Input: dimensioned drawing with shaded views. Units: mm. Origin: part minimum x, y, z. A direction names the side the tool comes from. Coordinates: 2 decimals unless noted, no trailing zeros. Write each loop counter-clockwise with the first axis right and the second up, starting at its lowest first coordinate (ties: lowest second). Pieces come first, ordered by that corner, then holes. Notation, with made-up numbers: (58.25, 23) -> (68.25, 23) arc R14 ccw to (68.25, 38) -> close; hole circle Ø7 at (19.5, 54). An arc over 180 degrees is marked (long way). One line per item, written item: value. Start each with the question number.
1. Line query: line 1 (X direction, y = 12, z = 9.75); line 2 (X direction, y = 2.25, z = 8.5); line 3 (Z direction, x = 23, y = 12.25). Output: solid intervals per line, ascending.
2. Access query for the marked faces 1 and 2. Directions: +Z, -Z, +X, -X, +Y, -Y. A direction counts if a zero-diameter tool reaches every point of the face in a straight line with its end or side. Return the directions, or none.
3. Section query B-B, the plane z = 12. Output: boundary loops of the cut face in (x, y), and give its area (3 significant figures).
4. Section query D-D, the plane x = 72. Output: boundary loops of the cut face in (y, z), and give its area (3 significant figures).
5. Section query C-C, the plane x = 102. Output: boundary loops of the cut face in (y, z), and give its area (3 significant figures).
6. Section query A-A, the plane y = 12. Output: boundary loops of the cut face in (x, z), and give its area (3 significant figures).
7. First-contact query: P1, Ø10, axis at x = 99, z = 17, coming from the +Y side; P2, Ø5, axis at x = 64.5, y = 11.5, coming from the -Z side; P3, Ø1.5, axis at x = 71.5, y = 6, coming from the +Z side. Flat tips, straight axial feed; report the tip coordinate or a pass-through.
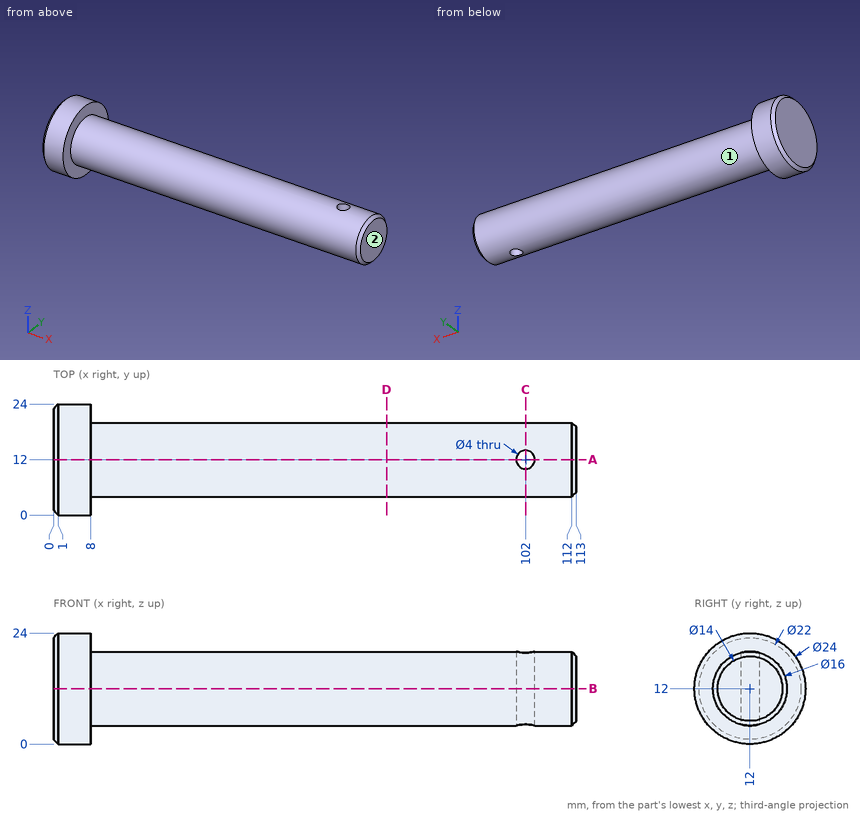
Computed values:
1. line 1: x = 0 to 100, 104 to 113
1. line 2: x = 0 to 8
1. line 3: z = 4 to 20
2. face 1: +X
2. face 2: +Z, -Z, +X, +Y, -Y
3. outline: (0, 1) -> (1, 0) -> (8, 0) -> (8, 4) -> (112, 4) -> (113, 5) -> (113, 19) -> (112, 20) -> (8, 20) -> (8, 24) -> (1, 24) -> (0, 23) -> close; hole circle Ø4 at (102, 12)
3. area: 1,860 mm²
4. outline: circle Ø16 at (12, 12)
4. area: 201 mm²
5. outline: (10, 4.25) -> (10, 19.75) arc R8 ccw to start; (14, 4.25) arc R8 ccw to (14, 19.75) -> close
5. area: 138 mm²
6. outline: (0, 1) -> (1, 0) -> (8, 0) -> (8, 4) -> (100, 4) -> (100, 20) -> (8, 20) -> (8, 24) -> (1, 24) -> (0, 23) -> close; (104, 4) -> (112, 4) -> (113, 5) -> (113, 19) -> (112, 20) -> (104, 20) -> close
6. area: 1,810 mm²
7. P1: stops at y = 20
7. P2: stops at z = 4
7. P3: stops at z = 18.04
